Input: part model. Units: mm. Frame: model coordinates. A direction names the side the tool comes from. Give positions to 0.01 mm unless a question says otherwise; leave off trailing zeros. Loops run counter-clockwise (first coordinate to the right, second up) from the corner with the lowest first, then second, coordinate; pieces in that order, holes last. Notation, with made-up numbers: (70, 80.5) - (74, 80.5) arc R15 ccw to (74, 109.5) - close; hole circle Ø11 at (1.5, -3). An arc over 180 degrees is marked (long way). Answer as a JSON object with one key per item and string values. Group by question number.
(1) Access query for faces 1 (the flat face through (8.2, 202, -14)), 2 (the flat face through (20, 202, 12)). Directions: +Z, -Z, +X, -X, +Y, -Y. A direction counts if a zero-diameter tool reaches every point of the face in a straight line with its end or side. Return the directions, or none.
(2) Material intervals for L1, parallel to X at y = 295, z = 8.5; L2, parallel to X at y = 312, z = 3, sorted ascending.
(3) Section query A-A (x = 12). Return loops of the section in (y, z), plus the area to 3 significant figures.
(4) Mould query, pull axis Z, two halves, no side actions, for faces 3 (the flat face through (14, 202, 19.05)), 4 (the flat face through (-12, 202, 20)), 5 (the flat face through (-14, 202, 8.2)), 6 (the flat face through (0, 410, -6)). Classes: +Z half, -Z half, draft (parallel to the pull), parting line (faces both ways), or undercut.
(5) Section query C-C (y = 227). Count the separate pieces of the cut face and the enclosed holes in it, plus the area to 3 significant figures.
(6) Section query B-B (z = 15.5). Return loops of the section in (x, y), plus the area to 3 significant figures.
(7) Pin query (flat end, axial travel): P1, Ø4, axis at x = 3.5, y = 351.5, coming from the -Z side. Return the tip coordinate at first contact, or that it passes through.
```python
from build123d import *

# Parameters (mm, degrees)
SKETCH1_W               = 10.85
SKETCH1_H               = 10.85
BOSS_EXTRUDE1_DEPTH     = 410
MIRROR2_COPY_1_SKETCH_W = 10.85
MIRROR2_COPY_1_SKETCH_H = 10.85
MIRROR2_COPY_1_DEPTH    = 410


with BuildPart() as part:
    # Sketch1 → Boss-Extrude1 (new body)
    with BuildSketch(Plane(origin=(0, 0, 0), x_dir=(1, 0, 0), z_dir=(0, 1, 0))):
        with BuildLine():
            Line((-4.3, 20), (-19.5, 20))
            ThreePointArc((-19.5, 20), (-19.853553391, 19.853553391), (-20, 19.5))
            Line((-20, 19.5), (-20, 4.3))
            Line((-20, 4.3), (-19.05, 4.3))
            Line((-19.05, 4.3), (-19.05, 7.25))
            Line((-19.05, 7.25), (-7.921751442, 7.25))
            Line((-7.921751442, 7.25), (-6.2, 5.528248558))
            Line((-6.2, 5.528248558), (-6.2, 0))
            Line((-6.2, 0), (-5.3, 0))
            ThreePointArc((-5.3, 0), (-5.066731596, 1.555066215), (-4.387460025, 2.973246463))
            Line((-4.387460025, 2.973246463), (-5.091168825, 3.676955262))
            ThreePointArc((-5.091168825, 3.676955262), (-5.091168825, 5.091168825), (-3.676955262, 5.091168825))
            Line((-3.676955262, 5.091168825), (-2.973246463, 4.387460025))
            ThreePointArc((-2.973246463, 4.387460025), (-1.555066215, 5.066731596), (0, 5.3))
            Line((0, 5.3), (0, 6.2))
            Line((0, 6.2), (-5.528248558, 6.2))
            Line((-5.528248558, 6.2), (-7.25, 7.921751442))
            Line((-7.25, 7.921751442), (-7.25, 19.05))
            Line((-7.25, 19.05), (-4.3, 19.05))
            Line((-4.3, 19.05), (-4.3, 20))
        make_face()
        with Locations((-13.625, 13.625)):
            Rectangle(SKETCH1_W, SKETCH1_H, mode=Mode.SUBTRACT)
    boss_extrude1 = extrude(amount=BOSS_EXTRUDE1_DEPTH)

    # Mirror1: Boss-Extrude1 across plane
    add(boss_extrude1.mirror(Plane(origin=(0, 0, 0), x_dir=(0, 0, 1), z_dir=(1, 0, 0))))

    # Mirror2: Boss-Extrude1 across plane
    add(boss_extrude1.mirror(Plane.XY))

    # Mirror2 copy 1 sketch → Mirror2 copy 1 (add)
    with BuildSketch(Plane(origin=(0, 0, 0), x_dir=(-1, 0, 0), z_dir=(0, 1, 0))):
        with BuildLine():
            Line((-4.3, 20), (-19.5, 20))
            ThreePointArc((-19.5, 20), (-19.853553391, 19.853553391), (-20, 19.5))
            Line((-20, 19.5), (-20, 4.3))
            Line((-20, 4.3), (-19.05, 4.3))
            Line((-19.05, 4.3), (-19.05, 7.25))
            Line((-19.05, 7.25), (-7.921751442, 7.25))
            Line((-7.921751442, 7.25), (-6.2, 5.528248558))
            Line((-6.2, 5.528248558), (-6.2, 0))
            Line((-6.2, 0), (-5.3, 0))
            ThreePointArc((-5.3, 0), (-5.066731596, 1.555066215), (-4.387460025, 2.973246463))
            Line((-4.387460025, 2.973246463), (-5.091168825, 3.676955262))
            ThreePointArc((-5.091168825, 3.676955262), (-5.091168825, 5.091168825), (-3.676955262, 5.091168825))
            Line((-3.676955262, 5.091168825), (-2.973246463, 4.387460025))
            ThreePointArc((-2.973246463, 4.387460025), (-1.555066215, 5.066731596), (0, 5.3))
            Line((0, 5.3), (0, 6.2))
            Line((0, 6.2), (-5.528248558, 6.2))
            Line((-5.528248558, 6.2), (-7.25, 7.921751442))
            Line((-7.25, 7.921751442), (-7.25, 19.05))
            Line((-7.25, 19.05), (-4.3, 19.05))
            Line((-4.3, 19.05), (-4.3, 20))
        make_face()
        with Locations((-13.625, 13.625)):
            Rectangle(MIRROR2_COPY_1_SKETCH_W, MIRROR2_COPY_1_SKETCH_H, mode=Mode.SUBTRACT)
    extrude(amount=MIRROR2_COPY_1_DEPTH)


solid = part.part
```
Recorded:
{
 "1": {"face 1": "+Y, -Y", "face 2": "+Z, -Z, +X, +Y, -Y"},
 "2": {"L1": "x = -20 to -19.05, -8.2 to -7.25, 7.25 to 8.2, 19.05 to 20", "L2": "x = -6.2 to -4.41, 4.41 to 6.2"},
 "3": {"outline": "(0, -20) - (410, -20) - (410, -19.05) - (0, -19.05) - close; (0, -8.2) - (410, -8.2) - (410, -7.25) - (0, -7.25) - close; (0, 7.25) - (410, 7.25) - (410, 8.2) - (0, 8.2) - close; (0, 19.05) - (410, 19.05) - (410, 20) - (0, 20) - close", "area": "1,560 mm^2"},
 "4": {"face 3": "undercut", "face 4": "+Z half", "face 5": "undercut", "face 6": "draft"},
 "5": {"separate pieces": "1", "enclosed holes": "5", "area": "261 mm^2"},
 "6": {"outline": "(-20, 0) - (-19.05, 0) - (-19.05, 410) - (-20, 410) - close; (-8.2, 0) - (-7.25, 0) - (-7.25, 410) - (-8.2, 410) - close; (7.25, 0) - (8.2, 0) - (8.2, 410) - (7.25, 410) - close; (19.05, 0) - (20, 0) - (20, 410) - (19.05, 410) - close", "area": "1,560 mm^2"},
 "7": {"P1": "stops at z = -20"}
}
